Read the model definition and answer for the solid it produces. Units are mm, in the model's axes. Give positions to 0.01 mm unless a question says otherwise; leave off trailing zeros. Write each loop counter-clockwise with the first axis right and the second up, starting at its lowest first coordinate (ties: lowest second). Pieces come first, ordered by that corner, then holes. Notation, with made-up numbers: M -8.5,8.5 L 21.5,8.5 A22 cw 21.5,37.5 Z; hole C -3.5,-18.5 d8. An arc over 180 degrees is marked long. Use a Markdown table: item, result. Add a question column.
Item 1: Consider probe 1 along X at (y, z) = (512.5, 21.75). Determine where the line is inside the solid, lowest interval first. Write a range as [from, to].
Item 2: A cutting plane is placed at C-C on z = 14.5. Determine the outline of the cut face in (x, y).
Item 3: A cutting plane is placed at A-A on y = 121. Determine the outline of the cut face in (x, z).
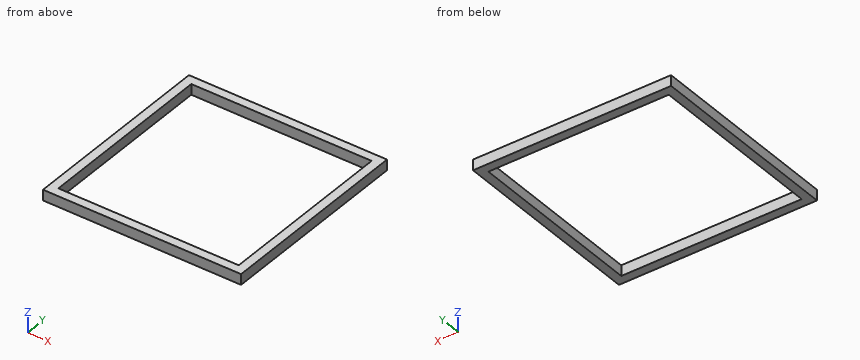
from build123d import *

# Parameters (mm, degrees)
SKETCH1_W           = 560
SKETCH1_H           = 560
SKETCH1_W_2         = 510
SKETCH1_H_2         = 510
BOSS_EXTRUDE1_DEPTH = 30


with BuildPart() as part:
    # Sketch1 → Boss-Extrude1 (new body)
    with BuildSketch(Plane.XY):
        with Locations((280, 280)):
            Rectangle(SKETCH1_W, SKETCH1_H)
        with Locations((280, 280)):
            Rectangle(SKETCH1_W_2, SKETCH1_H_2, mode=Mode.SUBTRACT)
    extrude(amount=BOSS_EXTRUDE1_DEPTH)


solid = part.part
Filled in:
| question | item | result |
|---|---|---|
| 1 | probe 1 | [0, 25], [535, 560] |
| 2 | outline | M 0,0 L 560,0 L 560,560 L 0,560 Z; hole M 25,25 L 535,25 L 535,535 L 25,535 Z |
| 3 | outline | M 0,0 L 25,0 L 25,30 L 0,30 Z; M 535,0 L 560,0 L 560,30 L 535,30 Z |
